Can you work these out from the model? Positions are in its coordinate system, mm. A direction names the side the tool comes from. Give positions to 0.01 mm unless a question says otherwise; leave off trailing zeros. Order: outer loops, then holes, each group sorted by start corner. A loop starts at its lowest first (then second) coordinate and runs counter-clockwise, first axis right, second up.
Item 1: I want a section at D-D, the plane z = -780. Write out the boundary of the cut face in (x, y), then the cut area to 3 significant figures.
Item 2: I want a section at B-B, the plane z = 176. Write out the boundary of the cut face in (x, y), then the cut area to 3 significant figures.
Item 3: If I drill on line 1 along Y through (x, z) = (113.5, 112); line 2 along Y through (x, z) = (60, -780); line 3 along Z through (x, y) = (46, 18.5), over which ranges is the centre line in solid material (lowest first)?
Item 4: Which directions (+Z, -Z, +X, -X, +Y, -Y) give clear straight access to the entire face, cutting with the end or side of a thin tool? Please do faces 4 (the flat face through (61, 0, -650)), 5 (the conical face through (115.24, -8.14, -799.62)).
Item 5: I want a section at A-A, the plane x = 32. Write out the boundary of the cut face in (y, z), then the cut area to 3 significant figures.
Item 6: If we mould it in two halves opening along Y, with no side actions, what happens to faces 1 (the flat face through (59, 60, 12)), 2 (the flat face through (120, 37, 12)), 3 (the flat face through (61, -25, 9))? For each: +Y half, -Y half, draft (parallel to the pull), parting line (faces both ways), or undercut.
Item 7: I want a section at C-C, the plane y = 0. Count the separate pieces of the cut face and the enclosed holes in it, then the cut area to 3 significant figures.
```python
from build123d import *

# Parameters (mm, degrees)
SKETCH_1_W          = 1660
SKETCH_1_H          = 120
EXTRUDE_1_DEPTH     = 120
SKETCH_2_W          = 1300
SKETCH_2_H          = 50
CUT_EXTRUDE_1_DEPTH = 841.773453434
SKETCH_3_R          = 21
CUT_EXTRUDE_2_DEPTH = 841.773453434
CHAMFER_1_SIZE      = 5


with BuildPart() as part:
    # 草图1 → 凸台-拉伸1 (new body)
    with BuildSketch(Plane(origin=(0, 0, 0), x_dir=(0, 0, -1), z_dir=(1, 0, 0))):
        Rectangle(SKETCH_1_W, SKETCH_1_H)
    extrude(amount=EXTRUDE_1_DEPTH)

    # 草图2 → 切除-拉伸1 (cut, through all)
    with BuildSketch(Plane(origin=(120, 0, 0), x_dir=(0, 0, -1), z_dir=(1, 0, 0))):
        Rectangle(SKETCH_2_W, SKETCH_2_H)
    extrude(amount=-CUT_EXTRUDE_1_DEPTH, mode=Mode.SUBTRACT)

    # 草图3 → 切除-拉伸2 (cut, through all)
    with BuildSketch(Plane(origin=(120, 0, 0), x_dir=(0, 0, -1), z_dir=(1, 0, 0))):
        with Locations((-780, 0)):
            Circle(SKETCH_3_R)
        with Locations((780, 0)):
            Circle(SKETCH_3_R)
    extrude(amount=-CUT_EXTRUDE_2_DEPTH, mode=Mode.SUBTRACT)

    # 倒角1
    chamfer_1_edges = [part.edges().sort_by_distance(p)[0] for p in [
        (120, 0, 830),
        (120, -60, 0),
        (0, 0, -650),
        (0, -25, 0),
        (0, 0, 650),
        (0, 25, 0),
        (120, 0, -650),
        (120, 25, 0),
        (120, 0, 650),
        (120, -25, 0),
        (0, 0, 801),
        (120, 0, 801),
        (0, 0, -759),
        (120, 0, -759),
        (120, 0, -830),
        (0, -60, 0),
        (0, 0, 830),
        (0, 60, 0),
        (0, 0, -830),
        (120, 60, 0),
        (60, -60, -830),
        (60, -60, 830),
        (60, 60, 830),
        (60, 60, -830),
    ]]
    chamfer(chamfer_1_edges, length=CHAMFER_1_SIZE)


solid = part.part
```
Results list:
1. outline: (0, -55) - (5, -60) - (115, -60) - (120, -55) - (120, -26) - (115, -21) - (5, -21) - (0, -26) - close; (0, 26) - (5, 21) - (115, 21) - (120, 26) - (120, 55) - (115, 60) - (5, 60) - (0, 55) - close
1. area: 9,260 mm2
2. outline: (0, -55) - (5, -60) - (115, -60) - (120, -55) - (120, -30) - (115, -25) - (5, -25) - (0, -30) - close; (0, 30) - (5, 25) - (115, 25) - (120, 30) - (120, 55) - (115, 60) - (5, 60) - (0, 55) - close
2. area: 8,300 mm2
3. line 1: y = -60 to -25, 25 to 60
3. line 2: y = -60 to -21, 21 to 60
3. line 3: z = -830 to -789.94, -770.06 to -650, 650 to 770.06, 789.94 to 830
4. face 4: +X, -X
4. face 5: +X
5. outline: (-60, -825) - (-55, -830) - (55, -830) - (60, -825) - (60, 825) - (55, 830) - (-55, 830) - (-60, 825) - close; hole (-25, -650) - (25, -650) - (25, 650) - (-25, 650) - close; hole circle Ø42 at (0, -780); hole circle Ø42 at (0, 780)
5. area: 131,000 mm2
6. face 1: +Y half
6. face 2: draft
6. face 3: undercut
7. separate pieces: 4
7. enclosed holes: 0
7. area: 32,900 mm2
